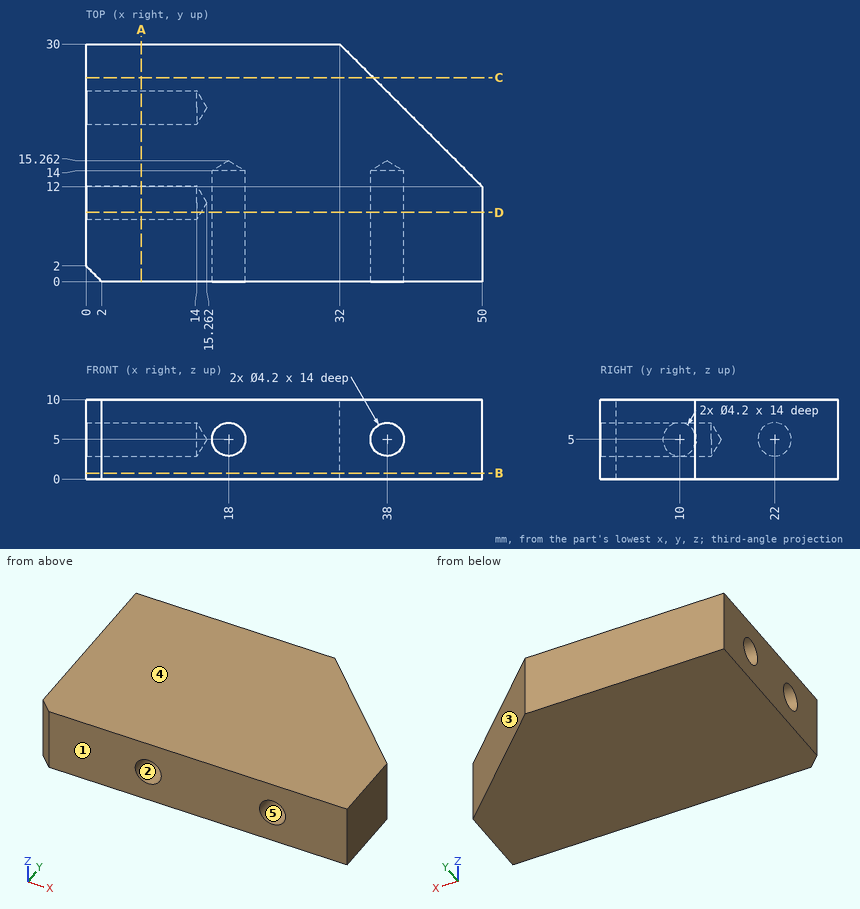
Here's the drawing with two shaded views (mm, measured from the low corner). I have some questions. A direction names the side the tool comes from. Give positions to 0.01 mm unless a question says otherwise; leave off trailing zeros. Loops run counter-clockwise (first coordinate to the right, second up) from the corner with the lowest first, then second, coordinate; pieces in that order, holes last. Notation, with made-up numbers: M 72.5,-20.5 L 113.5,-20.5 A20 cw 113.5,-14.5 Z; hole C 83.25,-17.75 d11. An arc over 180 degrees is marked long. Use one line per item in the form item = value. Start each with the question number.
Q1. If we section it at A-A (x = 7): Write out the boundary of the cut face in (y, z), then the cut area to 3 significant figures.
Q2. If we section it at B-B (z = 0.75): Write out the boundary of the cut face in (x, y).
Q3. I need wall thicknesses on line 1 along Y through (x, z) = (5, 5); line 2 along Y through (x, z) = (15, 5.25) (1 decimal); line 3 along Z through (x, y) = (8.75, 10). Which ranges of each line are inside material? Lowest first, please.
Q4. If we section it at D-D (y = 8.75): State how many separate pieces and enclosed holes the cut face has, then the cut area to 3 significant figures.
Q5. If we section it at C-C (y = 25.75): Write out the boundary of the cut face in (x, z), then the cut area to 4 significant figures.
Q6. Thinking about a two-plate mould opening in X: for the marked faces 3, 4 and 5, which applies, +X half, -X half, draft (parallel to the pull), parting line (faces both ways), or undercut?
Q7. Which directions (+Z, -Z, +X, -X, +Y, -Y) give clear straight access to the entire face, cutting with the end or side of a thin tool? Please do the marked faces 1 and 2.
Q8. Will this pin go through, and if not, where does the flat tip stop? pin 1 Ø1 at (y, z) = (20, 4) entering from +X.
Taken from the geometry:
q1.outline = M 0,0 L 30,0 L 30,10 L 0,10 Z; hole C 10,5 d4.2; hole C 22,5 d4.2
q1.area = 272 mm^2
q2.outline = M 0,2 L 2,0 L 50,0 L 50,12 L 32,30 L 0,30 Z
q3.line_1 = 0 to 7.9, 12.1 to 19.9, 24.1 to 30
q3.line_2 = 0 to 9.6, 10.4 to 21.6, 22.4 to 30
q3.line_3 = 0 to 2.9, 7.1 to 10
q4.separate_pieces = 1
q4.enclosed_holes = 2
q4.area = 424 mm^2
q5.outline = M 0,0 L 36.25,0 L 36.25,10 L 0,10 Z
q5.area = 362.5 mm^2
q6.face_3 = +X half
q6.face_4 = draft
q6.face_5 = undercut
q7.face_1 = +Z, -Z, +X, -X, -Y
q7.face_2 = -Y
q8.pin_1 = 42.5
